Model file for the job. Use its own axes, mm. Face numbers are marked on the shaded views. A direction names the side the tool comes from. Round coordinates to 2 decimals unless told otherwise and drop trailing zeros. Loops run counter-clockwise (first coordinate to the right, second up) from the corner with the lowest first, then second, coordinate; pieces in that order, holes last. Notation, with made-up numbers: M 33,26 L 92,26 A38 cw 92,65 Z; hole C 38,40.5 d6. An arc over 180 degrees is marked long. Use a Markdown table: item, result. Add a question column.
Q1. Cut at A-A (z = 0). Give the cut face in (x, y).
Q2. Tool access for the marked faces 5, 6 and 7: list every direction of +Z, -Z, +X, -X, +Y, -Y with a clear straight run to the whole face (end or side of a thin tool).
Q3. Probe line 1 (X direction, y = -38, z = 0); line 2 (Z direction, x = 40, y = -9); line 3 (Z direction, x = -6.5, y = -18). List the from-to ranges inside material, lowest first. Write a range as from..to.
Q4. Mould opens along X. For the marked faces 1, 2, 3 and 4 say: +X half, -X half, draft (parallel to the pull), parting line (faces both ways), or undercut.
Q5. Pin check, flat tips, straight feed: pin 1 (2 mm diameter, centred on y = -31, z = 3, fed in from -X); pin 2 (8 mm diameter, centred on y = -9.5, z = -36, fed in from +X); pin 3 (5 mm diameter, centred on x = 40.5, y = -4, fed in from -Z). Stop position of each tip, or through.
Q6. Cut at C-C (y = -12). Give the cut face in (x, z), plus the area to 3 significant figures.
Q7. Cut at B-B (x = 0). Give the cut face in (y, z), plus the area to 3 significant figures.
Q8. Cut at D-D (y = -29). Give the cut face in (x, z), plus the area to 3 significant figures.
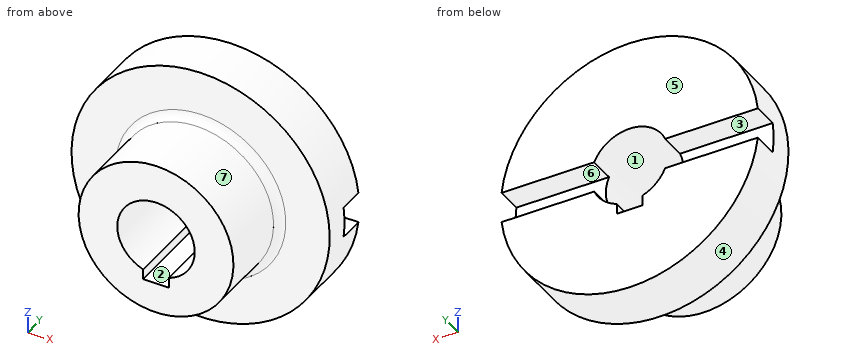
from build123d import *

# Parameters (mm, degrees)
BORE_KEYWAY_4MM_DEPTH  = 87.602540378
CROSS_SLOT_SKETCH_W    = 119.375340358
CROSS_SLOT_SKETCH_H    = 12
CROSS_SLOT_12X10_DEPTH = 10


with BuildPart() as part:
    # Flange Profile Sketch → Flange Body Revolve (revolve)
    with BuildSketch(Plane.XY, mode=Mode.PRIVATE) as flange_body_revolve_sk:
        with BuildLine():
            Line((0, 0), (50, 0))
            Line((50, 0), (50, -20))
            Line((50, -20), (33, -20))
            ThreePointArc((33, -20), (30.878679656, -20.878679656), (30, -23))
            Line((30, -23), (30, -50))
            Line((30, -50), (0, -50))
            Line((0, -50), (0, 0))
        make_face()
    revolve(flange_body_revolve_sk.sketch.rotate(Axis((0, 54.118773946, 0), (0, -1, 0)), 90), axis=Axis((0, 54.118773946, 0), (0, -1, 0)))

    # Bore Keyway Sketch → Bore Keyway 4mm (cut, through all)
    with BuildSketch(Plane(origin=(0, 0, 0), x_dir=(1, 0, 0), z_dir=(0, 1, 0))):
        with BuildLine():
            Line((-5, 14.142135624), (-5, 18.142135624))
            Line((-5, 18.142135624), (5, 18.142135624))
            Line((5, 18.142135624), (5, 14.142135624))
            ThreePointArc((5, 14.142135624), (0, -15), (-5, 14.142135624))
        make_face()
    extrude(amount=-BORE_KEYWAY_4MM_DEPTH, mode=Mode.SUBTRACT)

    # Cross Slot Sketch → Cross Slot 12x10 (cut)
    with BuildSketch(Plane(origin=(0, 0, 0), x_dir=(1, 0, 0), z_dir=(0, 1, 0))):
        Rectangle(CROSS_SLOT_SKETCH_W, CROSS_SLOT_SKETCH_H)
    extrude(amount=-CROSS_SLOT_12X10_DEPTH, mode=Mode.SUBTRACT)


solid = part.part
Checked values:
| question | item | result |
|---|---|---|
| 1 | outline | M -50,-20 L -33,-20 A3 cw -30,-23 L -30,-50 L -15,-50 L -15,-10 L -50,-10 Z; M 15,-50 L 30,-50 L 30,-23 A3 cw 33,-20 L 50,-20 L 50,-10 L 15,-10 Z |
| 2 | face 5 | +Z, -Z, +X, -X, +Y |
| 2 | face 6 | +X, -X, +Y |
| 2 | face 7 | -Y |
| 3 | line 1 | x = -30..-15, 15..30 |
| 3 | line 2 | z = -30..-6, 6..30 |
| 3 | line 3 | z = -49.58..-13.52, 13.52..49.58 |
| 4 | face 1 | undercut |
| 4 | face 2 | undercut |
| 4 | face 3 | draft |
| 4 | face 4 | parting line |
| 5 | pin 1 | stops at x = -29.93 |
| 5 | pin 2 | stops at x = 38.42 |
| 5 | pin 3 | stops at z = -32.5 |
| 6 | outline | C 0,0 d100; hole M -5,-18.14 L 5,-18.14 L 5,-14.14 A15 ccw long -5,-14.14 Z |
| 6 | area | 7,110 mm^2 |
| 7 | outline | M -50,-30 L -23,-30 A3 cw -20,-33 L -20,-50 L 0,-50 L 0,-18.14 L -50,-18.14 Z; M -50,15 L 0,15 L 0,50 L -20,50 L -20,33 A3 cw -23,30 L -50,30 Z |
| 7 | area | 2,150 mm^2 |
| 8 | outline | C 0,0 d60; hole M -5,-18.14 L 5,-18.14 L 5,-14.14 A15 ccw long -5,-14.14 Z |
| 8 | area | 2,090 mm^2 |
